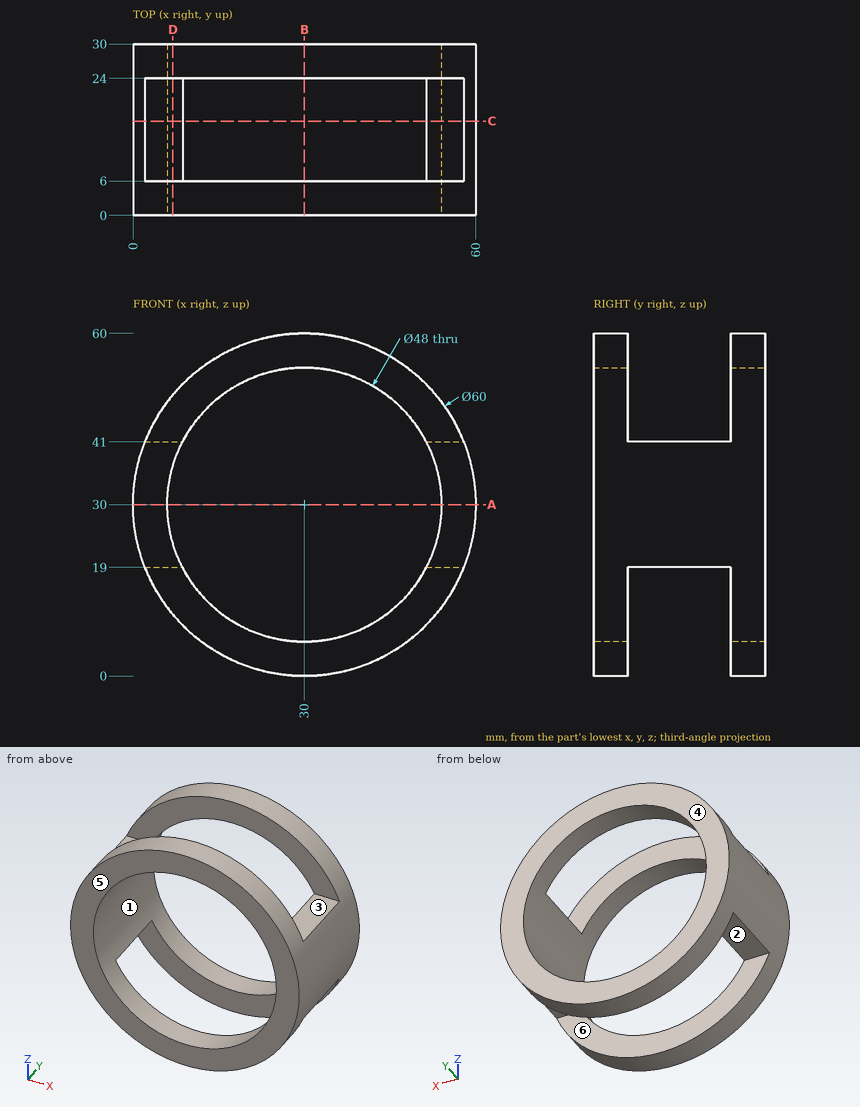
Verification items for this drawing (mm, ordinates from the low corner). A direction names the side the tool comes from. Coordinates: 2 decimals unless noted, no trailing zeros. Loops run counter-clockwise (first coordinate to the right, second up) from the corner with the lowest first, then second, coordinate; pieces in that order, holes last.
Item 1: Sectioned sample at A-A, the plane z = 30. Record the boundary of the cut face in (x, y).
Item 2: Thickness scan on line 1 (X direction, y = 11.75, z = 30); line 2 (Y direction, x = 52.5, z = 44.5); line 3 (Z direction, x = 3, y = 20.5). Record the ranges inside material, lowest first.
Item 3: Release check for a two-part mould opening along Y. For the marked faces 4, 5 and 6 record: released by +Y, released by -Y, zero draft, split by the parting line, or undercut.
Item 4: Sectioned sample at C-C, the plane y = 16.5. Record the boundary of the cut face in (x, z), then the cut area to 3 significant figures.
Item 5: Access from +Z, -Z, +X, -X, +Y, -Y to the whole of each face (thin tool, end or side, straight path). Record for the marked faces 1, 2 and 3.
Item 6: Sectioned sample at D-D, the plane x = 7. Record the boundary of the cut face in (y, z), then the cut area to 3 significant figures.
Item 7: Sectioned sample at B-B, the plane x = 30. Record the boundary of the cut face in (y, z).
Item 8: Go/stop test with flat-tipped pins: pin 1 Ø5.5 at (x, y) = (55, 11) entering from +Z; pin 2 Ø3.5 at (x, y) = (54, 12.5) entering from -Z; pin 3 Ø8 at (y, z) = (6, 45.5) entering from +X; pin 4 Ø12 at (x, y) = (27, 10.5) entering from -Z. Record where each tip stops, or that it passes through.
Check result:
1. outline: (0, 0) - (6, 0) - (6, 30) - (0, 30) - close; (54, 0) - (60, 0) - (60, 30) - (54, 30) - close
2. line 1: x = 0 to 6, 54 to 60
2. line 2: y = 0 to 6, 24 to 30
2. line 3: z = 19 to 41
3. face 4: released by +Y
3. face 5: released by -Y
3. face 6: undercut
4. outline: (2.09, 19) - (8.67, 19) arc R24 cw to (8.67, 41) - (2.09, 41) arc R30 ccw to start; (51.33, 19) - (57.91, 19) arc R30 ccw to (57.91, 41) - (51.33, 41) arc R24 cw to start
4. area: 272 mm2
5. face 1: +Y, -Y
5. face 2: -Z, +X, -X
5. face 3: +Z, +X, -X
6. outline: (0, 10.74) - (6, 10.74) - (6, 19) - (24, 19) - (24, 10.74) - (30, 10.74) - (30, 23.14) - (0, 23.14) - close; (0, 36.86) - (30, 36.86) - (30, 49.26) - (24, 49.26) - (24, 41) - (6, 41) - (6, 49.26) - (0, 49.26) - close
6. area: 447 mm2
7. outline: (0, 0) - (6, 0) - (6, 6) - (0, 6) - close; (0, 54) - (6, 54) - (6, 60) - (0, 60) - close; (24, 0) - (30, 0) - (30, 6) - (24, 6) - close; (24, 54) - (30, 54) - (30, 60) - (24, 60) - close
8. pin 1: stops at z = 41
8. pin 2: stops at z = 19
8. pin 3: stops at x = 57.71
8. pin 4: stops at z = 0
